Geometry: final body of the model. Coordinates: model frame, mm. A direction names the side the tool comes from. Coordinates: 2 decimals unless noted, no trailing zeros. Order: outer loops, then holes, each group sorted by start corner. A loop starts at its lowest first (then second) coordinate and runs counter-clockwise, first axis right, second up. Notation, with made-up numbers: M 17.25,42.25 L 71.25,42.25 A9 ccw 71.25,52.25 Z; hole C 86,-32.5 d3. An arc over 180 degrees is marked long. Write item = value, one per line. Start each with the question number.
```python
from build123d import *

# Parameters (mm, degrees)
SKETCH1_W                    = 480
SKETCH1_H                    = 220
BOSS_EXTRUDE1_DEPTH          = 120
CUT_EXTRUDE1_DEPTH           = 291
CUT_EXTRUDE1_DEPTH_BACK      = 291
SKETCH2_R                    = 140
CUT_EXTRUDE2_DEPTH           = 291
CUT_EXTRUDE2_DEPTH_BACK      = 291
SKETCH4_R                    = 12.5
M16_TAPPED_HOLE1_D           = 14
M16_TAPPED_HOLE1_DEPTH       = 32
M16_TAPPED_HOLE1_CSINK_D     = 16.05
M16_TAPPED_HOLE1_CSINK_ANGLE = 100
M16_TAPPED_HOLE1_TIP         = 4.206024333


with BuildPart() as part:
    # Sketch1 → Boss-Extrude1 (new body)
    with BuildSketch(Plane.XY):
        Rectangle(SKETCH1_W, SKETCH1_H)
    extrude(amount=BOSS_EXTRUDE1_DEPTH)

    # Sketch2 → Cut-Extrude1 (cut, two sides: drawn at the far end of the back side and taken through both)
    with BuildSketch(Plane.XY.offset(120).offset(-CUT_EXTRUDE1_DEPTH_BACK)):
        with Locations((0, 110)):
            Circle(SKETCH2_R)
    extrude(amount=CUT_EXTRUDE1_DEPTH + CUT_EXTRUDE1_DEPTH_BACK, mode=Mode.SUBTRACT)

    # Sketch4 → Cut-Extrude2 (cut, two sides: drawn at the far end of the back side and taken through both)
    with BuildSketch(Plane.XY.offset(120).offset(-CUT_EXTRUDE2_DEPTH_BACK)):
        with Locations((0, -70)):
            Circle(SKETCH4_R)
        with Locations((-31.25667198, -67.265395542)):
            Circle(SKETCH4_R)
        with Locations((31.25667198, -67.265395542)):
            Circle(SKETCH4_R)
    extrude(amount=CUT_EXTRUDE2_DEPTH + CUT_EXTRUDE2_DEPTH_BACK, mode=Mode.SUBTRACT)

    # M16 Tapped Hole1
    with Locations(Plane.XY.offset(120)):
        with Locations((-166.298315852, 41.116982174), (166.298315852, 41.116982174), (68.883017826, -56.298315852), (-75.868170831, -53.229962491)):
            CounterSinkHole(M16_TAPPED_HOLE1_D / 2, M16_TAPPED_HOLE1_CSINK_D / 2, depth=M16_TAPPED_HOLE1_DEPTH, counter_sink_angle=M16_TAPPED_HOLE1_CSINK_ANGLE)
            with Locations((0, 0, -(M16_TAPPED_HOLE1_DEPTH + M16_TAPPED_HOLE1_TIP / 2))):  # 118° drill point
                Cone(0, M16_TAPPED_HOLE1_D / 2, M16_TAPPED_HOLE1_TIP, mode=Mode.SUBTRACT)


solid = part.part
```
Item 1: Section query C-C on z = 97. Output: boundary loops of the cut face in (x, y).
Item 2: Section query D-D on z = 31. Output: boundary loops of the cut face in (x, y).
Item 3: Material intervals for probe 1 along X at (y, z) = (-64.5, 84); probe 2 along X at (y, z) = (43, 13); probe 3 along X at (y, z) = (-13, 65), sorted ascending. Write a range as [from, to].
Item 4: Section query B-B on y = 63. Output: boundary loops of the cut face in (x, z).
Item 5: Reachability of faces 1 (the cylindrical face through (-82.545, -51.127, 103.352)), 2 (the cylindrical face through (-19.334, -63.511, 59.16)) from +Z, -Z, +X, -X, +Y, -Y: full face, straight path, thin tool, end or side. Return the list, or none.
Item 6: Draft query along Y for faces 3 (the cylindrical face through (-161.14, 45.85, 103.35)), 4 (the cylindrical face through (-3.079, -29.966, 59.16)), 5 (the flat face through (240, -2, 59)). Return one class per face: pulls with the +Y half, pulls with the -Y half, needs draft (parallel to the pull), parting line crosses it, or undercut.
Item 7: Section query A-A on x = 0. Output: boundary loops of the cut face in (y, z).
Ans:
q1.outline = M -240,-110 L 240,-110 L 240,110 L 140,110 A140 cw -140,110 L -240,110 Z; hole C -166.3,41.12 d14; hole C -75.87,-53.23 d14; hole C -31.26,-67.27 d25; hole C 0,-70 d25; hole C 31.26,-67.27 d25; hole C 68.88,-56.3 d14; hole C 166.3,41.12 d14
q2.outline = M -240,-110 L 240,-110 L 240,110 L 140,110 A140 cw -140,110 L -240,110 Z; hole C -31.26,-67.27 d25; hole C 0,-70 d25; hole C 31.26,-67.27 d25
q3.probe_1 = [-240, -43.45], [-19.07, -11.22], [11.22, 19.07], [43.45, 240]
q3.probe_2 = [-240, -122.93], [122.93, 240]
q3.probe_3 = [-240, -66.87], [66.87, 240]
q4.outline = M -240,0 L -131.87,0 L -131.87,120 L -240,120 Z; M 131.87,0 L 240,0 L 240,120 L 131.87,120 Z
q5.face_1 = +Z
q5.face_2 = +Z, -Z
q6.face_3 = undercut
q6.face_4 = pulls with the +Y half
q6.face_5 = needs draft
q7.outline = M -110,0 L -82.5,0 L -82.5,120 L -110,120 Z; M -57.5,0 L -30,0 L -30,120 L -57.5,120 Z
